from build123d import *

# Parameters (mm, degrees)
SKETCH1_W      = 38.1
SKETCH1_H      = 38.1
BASEHEAD_DEPTH = 17.3736


with BuildPart() as part:
    # Sketch1 → BaseHead (new body)
    with BuildSketch(Plane(origin=(0, 0, 0), x_dir=(0, 0.7071067811865488, -0.7071067811865462), z_dir=(1, 0, 0))):
        Rectangle(SKETCH1_W, SKETCH1_H)
    extrude(amount=BASEHEAD_DEPTH)

    # BodySke → Body (revolve)
    with BuildSketch(Plane.XY, mode=Mode.PRIVATE) as body_sk:
        Polygon((17.3736, 0), (17.3736, 12.7), (91.6813, 12.7), (93.5736, 10.8077), (93.5736, 0), align=None)
    revolve(body_sk.sketch.rotate(Axis((0, 0, 0), (1, 0, 0)), 90), axis=Axis((0, 0, 0), (1, 0, 0)))

    # Sketch3 → HeadChamfer (revolve, cut)
    with BuildSketch(Plane.XY):
        Polygon((0, 19.05), (-12.7, 19.05), (-12.7, 52.340768363), (15.523740234, 52.340768363), align=None)
    revolve(axis=Axis((0, 0, 0), (1, 0, 0)), mode=Mode.SUBTRACT)


solid = part.part
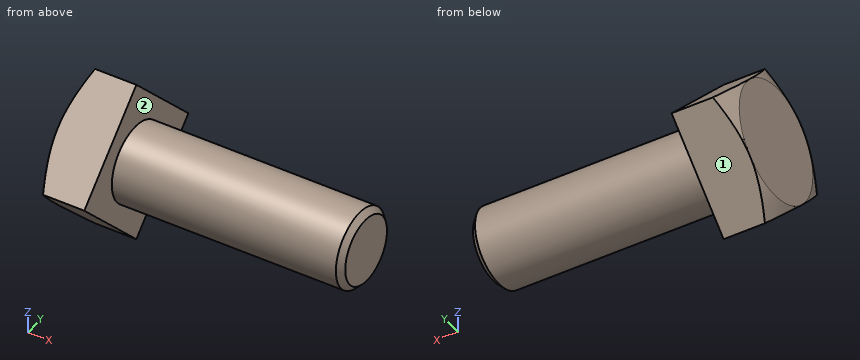
Check sheet for the modelled part. Datum: model origin and axes. Units: mm. Face numbers are marked on the shaded views. A direction names the side the tool comes from. Coordinates: 2 decimals unless noted, no trailing zeros. Write each loop counter-clockwise with the first axis right and the second up, starting at its lowest first coordinate (ties: lowest second). Pieces come first, ordered by that corner, then holes.
Item 1: Cross-section at A-A on x = 14. Record the boundary of the cut face in (y, z).
Numbers:
outline: (-26.94, 0) - (0, -26.94) - (26.94, 0) - (0, 26.94) - close
Item 2: Scan lines: probe 1 along X at (y, z) = (16, -2); probe 2 along Y at (x, z) = (68, -7); probe 3 along Y at (x, z) = (10.5, -12.5). Record each from-to range of solid material in increasing order.
Numbers:
probe 1: x = 0 to 17.37
probe 2: y = -10.6 to 10.6
probe 3: y = -14.44 to 14.44
Item 3: Access from +Z, -Z, +X, -X, +Y, -Y to the whole of each face (thin tool, end or side, straight path). Record for the marked faces 1 and 2.
Numbers:
face 1: -Z, +X, -X, +Y
face 2: +X
Item 4: Depth check by flat-ended pin: pin 1 Ø10 at (x, y) = (25.5, -2.5) entering from -Z; pin 2 Ø2 at (x, z) = (60, 3.5) entering from -Y; pin 3 Ø2 at (y, z) = (3.5, -20) entering from -X. Enter the tip coordinate at first touch or a pass-through.
Numbers:
pin 1: stops at z = -12.7
pin 2: stops at y = -12.45
pin 3: stops at x = 0.12
Item 5: Cross-section at B-B on x = 86. Record the boundary of the cut face in (y, z), then the cut area to 3 significant figures.
Numbers:
outline: circle Ø25.4 at (0, 0)
area: 507 mm2
